from build123d import *

# Parameters (mm, degrees)
RAIL_PROFILE_SKETCH_W           = 580
RAIL_PROFILE_SKETCH_H           = 60
RAIL_BAR_580X60X28_DEPTH        = 28
EDGE_FILLET_R5_R                = 5
GROOVE_SKETCH_W                 = 16
GROOVE_SKETCH_H                 = 16
LONGITUDINAL_GROOVE_16X16_DEPTH = 582.449911858
EDGE_CHAMFER_10X45_SIZE         = 10
MOUNTING_HOLES_SKETCH_R         = 6.25
MOUNTING_HOLES_5X_DEPTH         = 293.889057494


with BuildPart() as part:
    # Rail Profile Sketch → Rail Bar 580x60x28 (new body)
    with BuildSketch(Plane.XY):
        Rectangle(RAIL_PROFILE_SKETCH_W, RAIL_PROFILE_SKETCH_H)
    extrude(amount=RAIL_BAR_580X60X28_DEPTH)

    # Edge Fillet R5
    edge_fillet_r5_edges = [part.edges().sort_by_distance(p)[0] for p in [
        (0, 30, 28),
    ]]
    fillet(edge_fillet_r5_edges, radius=EDGE_FILLET_R5_R)

    # Groove Sketch → Longitudinal Groove 16x16 (cut, through all)
    with BuildSketch(Plane(origin=(290, 0, 0), x_dir=(0, 0, -1), z_dir=(1, 0, 0))):
        with Locations((0, -7)):
            Rectangle(GROOVE_SKETCH_W, GROOVE_SKETCH_H)
    extrude(amount=-LONGITUDINAL_GROOVE_16X16_DEPTH, mode=Mode.SUBTRACT)

    # Edge Chamfer 10x45
    edge_chamfer_10x45_edges = [part.edges().sort_by_distance(p)[0] for p in [
        (0, 30, 0),
    ]]
    chamfer(edge_chamfer_10x45_edges, length=EDGE_CHAMFER_10X45_SIZE)

    # Mounting Holes Sketch → Mounting Holes 5x (cut, through all)
    with BuildSketch(Plane.XY.offset(28)):
        with Locations((-265, -7)):
            Circle(MOUNTING_HOLES_SKETCH_R)
        with Locations((-132.5, -7)):
            Circle(MOUNTING_HOLES_SKETCH_R)
        with Locations((0, -7)):
            Circle(MOUNTING_HOLES_SKETCH_R)
        with Locations((132.5, -7)):
            Circle(MOUNTING_HOLES_SKETCH_R)
        with Locations((265, -7)):
            Circle(MOUNTING_HOLES_SKETCH_R)
    extrude(amount=-MOUNTING_HOLES_5X_DEPTH, mode=Mode.SUBTRACT)


solid = part.part
Model file for the job. Use its own axes, mm. A direction names the side the tool comes from. Round coordinates to 2 decimals unless told otherwise and drop trailing zeros. Order: outer loops, then holes, each group sorted by start corner. A loop starts at its lowest first (then second) coordinate and runs counter-clockwise, first axis right, second up.
(1) Band-saw the part on A-A (y = -7). List the corners of the cut face in (x, z).
(2) Drill centre lines: line 1 (X direction, y = -2.5, z = 8.75); line 2 (Y direction, x = 265, z = 18.5); line 3 (Y direction, x = 132.5, z = 24.25). Where is each one in solid material? Low to high.
(3) Pin check, flat tips, straight feed: pin 1 (6.5 mm diameter, centred on x = -136.5, z = 3.5, fed in from +Y); pin 2 (14.5 mm diameter, centred on x = -132.5, y = -7, fed in from -Z); pin 3 (10 mm diameter, centred on x = 132.5, y = -7, fed in from -Z) (3 decimals). Stop position of each tip, or through.
(4) 3-axis set-ups, long thin cutter, end or side, ignore diameter. For faces 4 (the face through (-60, -7, 8)), 5 (the face through (-271.244, -6.725, 18.14)): which of +Z, -Z, +X, -X, +Y, -Y reach the whole face in a straight line?
(5) Band-saw the part on C-C (x = -12). List the corners of the cut face in (y, z).
(6) Pull direction X, two halves, no side cores. Call faces 1 (the face through (290, 0, 14)), 2 (the face through (-4, 25, 5)), 3 (the face through (-126.54, -5.12, 18.14)): released by +X, released by -X, zero draft, split by the parting line, or undercut.
(7) Band-saw the part on B-B (x = -132.5). List the corners of the cut face in (y, z).
Verdict:
1. outline: (-290, 8) - (-271.25, 8) - (-271.25, 28) - (-290, 28) - close; (-258.75, 8) - (-138.75, 8) - (-138.75, 28) - (-258.75, 28) - close; (-126.25, 8) - (-6.25, 8) - (-6.25, 28) - (-126.25, 28) - close; (6.25, 8) - (126.25, 8) - (126.25, 28) - (6.25, 28) - close; (138.75, 8) - (258.75, 8) - (258.75, 28) - (138.75, 28) - close; (271.25, 8) - (290, 8) - (290, 28) - (271.25, 28) - close
2. line 1: x = -290 to -269.34, -260.66 to -136.84, -128.16 to -4.34, 4.34 to 128.16, 136.84 to 260.66, 269.34 to 290
2. line 2: y = -30 to -13.25, -0.75 to 30
2. line 3: y = -30 to -13.25, -0.75 to 29.84
3. pin 1: stops at y = 26.75
3. pin 2: stops at z = 8
3. pin 3: passes through
4. face 4: -Z, +X, -X
4. face 5: +Z, -Z
5. outline: (-30, 0) - (-15, 0) - (-15, 8) - (1, 8) - (1, 0) - (20, 0) - (30, 10) - (30, 23) arc R5 ccw to (25, 28) - (-30, 28) - close
6. face 1: released by +X
6. face 2: zero draft
6. face 3: undercut
7. outline: (-30, 0) - (-15, 0) - (-15, 8) - (-13.25, 8) - (-13.25, 28) - (-30, 28) - close; (-0.75, 8) - (1, 8) - (1, 0) - (20, 0) - (30, 10) - (30, 23) arc R5 ccw to (25, 28) - (-0.75, 28) - close
